Geometry: final body of the model. Coordinates: model frame, mm. Face numbers are marked on the shaded views. A direction names the side the tool comes from. Give positions to 0.01 mm unless a question says otherwise; leave off trailing zeros. Write each loop counter-clockwise with the first axis right and the second up, starting at its lowest first coordinate (ties: lowest second). Pieces come first, ordered by that corner, then holes. Notation, with made-up numbers: (-21.5, 37.25) -> (6.5, 37.25) arc R17 ccw to (6.5, 59.25) -> close; hole circle Ø1 at (8, 44). An arc over 180 degrees is marked (long way). Use CSV: the item, a comma, the result in double quotes. Start each with the question number.
1) Section D-D (y = -37). Output: boundary loops of the cut face in (x, z).
2) Section C-C (z = 28.5). Output: boundary loops of the cut face in (x, y).
3) Section B-B (x = 210). Output: boundary loops of the cut face in (y, z).
4) Set-up query: the marked faces 1, 2 and 3. Return all of +Z, -Z, +X, -X, +Y, -Y with unobstructed straight access to the full face (end or side cutting, diameter ignored); none if empty.
5) Material intervals for line 1 (Z direction, x = 210, y = -37.25); line 2 (X direction, y = -36.35, z = 20); line 3 (X direction, y = -38.05, z = 20), sorted ascending. Write a range as [from, to].
6) Contact query for flat-ended pins moving along their axis: P1, Ø20, axis at y = -13, z = 28, coming from the -X side; P2, Ø9, axis at x = 140, z = 20, coming from the +Y side; P3, Ø8, axis at x = 210, z = 20, coming from the -Y side; P4, Ø6, axis at y = -19, z = 11.5, coming from the -X side. Output: stop coordinate, or through.
7) Section A-A (z = 20). Output: boundary loops of the cut face in (x, y).
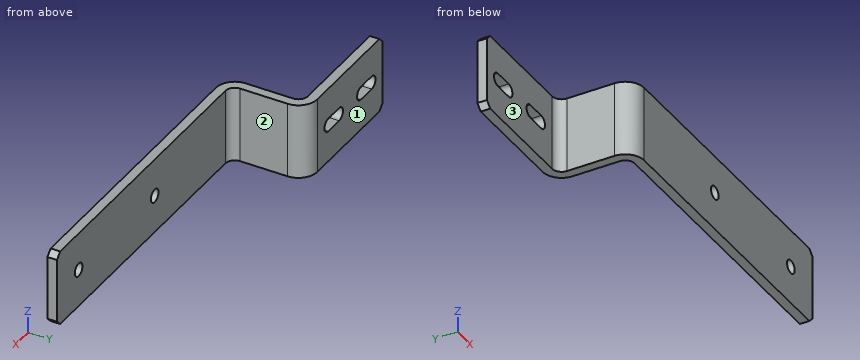
```python
from build123d import *

# Parameters (mm, degrees)
BOSS_EXTRUDE1_DEPTH = 40
CUT_EXTRUDE1_DEPTH  = 40
SKETCH3_R           = 3.5
CUT_EXTRUDE2_DEPTH  = 40
CHAMFER1_SIZE       = 3


with BuildPart() as part:
    # Sketch1 → Boss-Extrude1 (new body)
    with BuildSketch(Plane.XY):
        with BuildLine():
            Line((0, 0), (60, 0))
            ThreePointArc((60, 0), (63.535533906, -1.464466094), (65, -5))
            Line((65, -5), (65, -30))
            ThreePointArc((65, -30), (67.928932188, -37.071067812), (75, -40))
            Line((75, -40), (230, -40))
            Line((230, -40), (230, -35))
            Line((230, -35), (75, -35))
            ThreePointArc((75, -35), (71.464466094, -33.535533906), (70, -30))
            Line((70, -30), (70, -5))
            ThreePointArc((70, -5), (67.071067812, 2.071067812), (60, 5))
            Line((60, 5), (0, 5))
            Line((0, 5), (0, 0))
        make_face()
    extrude(amount=BOSS_EXTRUDE1_DEPTH)

    # Sketch2 → Cut-Extrude1 (cut)
    with BuildSketch(Plane(origin=(0, 5, 0), x_dir=(1, 0, 0), z_dir=(0, 1, 0))):
        with BuildLine():
            Line((10, -16.5), (20, -16.5))
            ThreePointArc((20, -16.5), (23.5, -20), (20, -23.5))
            Line((20, -23.5), (10, -23.5))
            ThreePointArc((10, -23.5), (6.5, -20), (10, -16.5))
        make_face()
        with BuildLine():
            Line((40, -16.5), (50, -16.5))
            ThreePointArc((50, -16.5), (53.5, -20), (50, -23.5))
            Line((50, -23.5), (40, -23.5))
            ThreePointArc((40, -23.5), (36.5, -20), (40, -16.5))
        make_face()
    extrude(amount=-CUT_EXTRUDE1_DEPTH, mode=Mode.SUBTRACT)

    # Sketch3 → Cut-Extrude2 (cut)
    with BuildSketch(Plane(origin=(0, -35, 0), x_dir=(1, 0, 0), z_dir=(0, 1, 0))):
        with Locations(Location((140, -20, 0), (0, 0, 270))):
            Circle(SKETCH3_R)
        with Locations(Location((210, -20, 0), (0, 0, 270))):
            Circle(SKETCH3_R)
    extrude(amount=-CUT_EXTRUDE2_DEPTH, mode=Mode.SUBTRACT)

    # Chamfer1
    chamfer1_edges = [part.edges().sort_by_distance(p)[0] for p in [
        (0, 2.5, 0),
        (230, -37.5, 0),
        (0, 2.5, 40),
        (230, -37.5, 40),
    ]]
    chamfer(chamfer1_edges, length=CHAMFER1_SIZE)


solid = part.part
```
Answers follow:
1,outline,"(67.86, 0) -> (227, 0) -> (230, 3) -> (230, 37) -> (227, 40) -> (67.86, 40) -> close; hole circle Ø7 at (140, 20); hole circle Ø7 at (210, 20)"
2,outline,"(0, 0) -> (60, 0) arc R5 cw to (65, -5) -> (65, -30) arc R10 ccw to (75, -40) -> (230, -40) -> (230, -35) -> (75, -35) arc R5 cw to (70, -30) -> (70, -5) arc R10 ccw to (60, 5) -> (0, 5) -> close"
3,outline,"(-40, 0) -> (-35, 0) -> (-35, 16.5) -> (-40, 16.5) -> close; (-40, 23.5) -> (-35, 23.5) -> (-35, 40) -> (-40, 40) -> close"
4,face 1,"+Z, -Z, +X, -X, +Y"
4,face 2,"+Z, -Z, +X, +Y"
4,face 3,"+Z, -Z, -X, -Y"
5,line 1,"z = [0, 16.5], [23.5, 40]"
5,line 2,"x = [67.27, 136.5], [143.5, 206.5], [213.5, 230]"
5,line 3,"x = [69.07, 136.5], [143.5, 206.5], [213.5, 230]"
6,P1,"stops at x = 64.58"
6,P2,"stops at y = -35"
6,P3,"stops at y = -40"
6,P4,"stops at x = 65"
7,outline,"(0, 0) -> (6.5, 0) -> (6.5, 5) -> (0, 5) -> close; (23.5, 0) -> (36.5, 0) -> (36.5, 5) -> (23.5, 5) -> close; (53.5, 0) -> (60, 0) arc R5 cw to (65, -5) -> (65, -30) arc R10 ccw to (75, -40) -> (136.5, -40) -> (136.5, -35) -> (75, -35) arc R5 cw to (70, -30) -> (70, -5) arc R10 ccw to (60, 5) -> (53.5, 5) -> close; (143.5, -40) -> (206.5, -40) -> (206.5, -35) -> (143.5, -35) -> close; (213.5, -40) -> (230, -40) -> (230, -35) -> (213.5, -35) -> close"
